CAD build for the part. Positions are in the model's coordinates, mm. Face numbers are marked on the shaded views. A direction names the side the tool comes from. Give positions to 0.01 mm unless a question says otherwise; leave off trailing zeros. Write each loop counter-clockwise with the first axis right and the second up, starting at its lowest first coordinate (ties: lowest second). Pieces come first, ordered by that corner, then holes. Notation, with made-up numbers: (3, -28) - (12, -28) arc R15 cw to (12, 0) - close; hole circle Ø10 at (46, -32.75). An arc over 180 degrees is marked (long way). Answer as a JSON object with one key per item and string values.
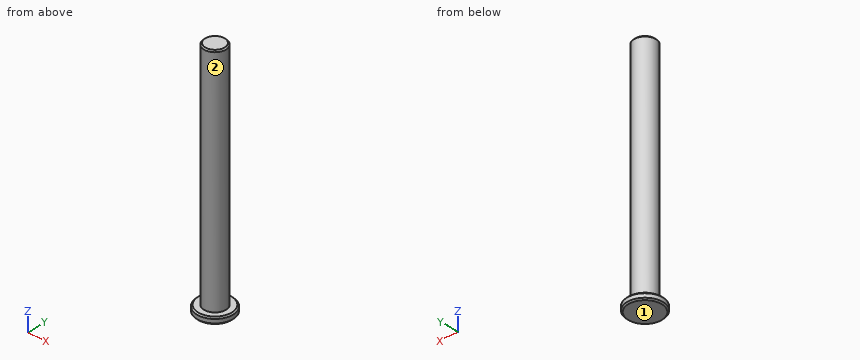
from build123d import *

# Parameters (mm, degrees)
SKETCH1_R           = 25
BOSS_EXTRUDE1_DEPTH = 526
SKETCH2_R           = 41
BOSS_EXTRUDE2_DEPTH = 15
CHAMFER1_SIZE       = 3


with BuildPart() as part:
    # Sketch1 → Boss-Extrude1 (new body)
    with BuildSketch(Plane.XY):
        Circle(SKETCH1_R)
    extrude(amount=BOSS_EXTRUDE1_DEPTH)

    # Sketch2 → Boss-Extrude2 (add)
    with BuildSketch(Plane(origin=(0, 0, 0), x_dir=(-1, 0, 0), z_dir=(0, 0, -1))):
        Circle(SKETCH2_R)
    extrude(amount=BOSS_EXTRUDE2_DEPTH)

    # Chamfer1
    chamfer1_edges = [part.edges().sort_by_distance(p)[0] for p in [
        (-25, 0, 526),
        (41, 0, 0),
        (41, 0, -15),
    ]]
    chamfer(chamfer1_edges, length=CHAMFER1_SIZE)


solid = part.part
Item 1: Which spindle directions (+Z, -Z, +X, -X, +Y, -Y) get a long thin tool onto all of the face, cutting with end or side? Do the marked faces 1 and 2. Say none if no direction does.
Entries:
{"face 1": "-Z, +X, -X, +Y, -Y", "face 2": "+Z"}
Item 2: Cut at A-A (y = 0). Give the cut face in (x, z), and give its area (3 significant figures).
Entries:
{"outline": "(-41, -12) - (-38, -15) - (38, -15) - (41, -12) - (41, -3) - (38, 0) - (25, 0) - (25, 523) - (22, 526) - (-22, 526) - (-25, 523) - (-25, 0) - (-38, 0) - (-41, -3) - close", "area": "27,500 mm2"}
Item 3: Flat gauge pins, fed straight in: P1, Ø3, axis at y = 10, z = 226, coming from the -X side; P2, Ø5, axis at y = 19, z = 355.5, coming from the +X side; P3, Ø12, axis at x = 21, y = -32.5, coming from the +Z side. Where does each tip first touch, or does it go through?
Entries:
{"P1": "x = -23.51", "P2": "x = 18.78", "P3": "z = 0"}
Item 4: Cut at C-C (z = 52). Give the cut face in (x, y).
Entries:
{"outline": "circle Ø50 at (0, 0)"}
Item 5: Probe line 1 (Z direction, x = -12, y = 24); line 2 (Y direction, x = 0, z = 12); line 3 (Y direction, x = -9, z = 282). List the from-to ranges inside material, lowest first. Write a range as from..to.
Entries:
{"line 1": "-15..0", "line 2": "-25..25", "line 3": "-23.32..23.32"}
